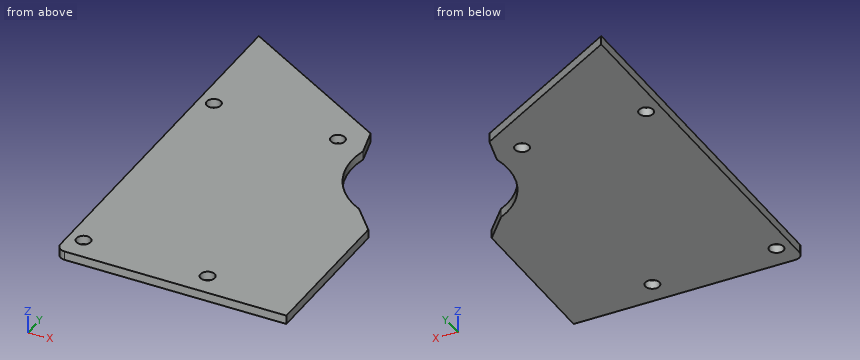
```python
from build123d import *

# Parameters (mm, degrees)
BOSS_EXTRUDE1_DEPTH        = 5
F_16_0_16_DIAMETER_HOLE1_D = 16
FILLET1_R                  = 10


with BuildPart() as part:
    # Sketch1 → Boss-Extrude1 (new, symmetric)
    with BuildSketch(Plane.XY):
        with BuildLine():
            Line((0, 0), (0, 436))
            Line((0, 436), (181, 331.499601277))
            Line((181, 331.499601277), (189.323079198, 299.499601277))
            ThreePointArc((189.323079198, 299.499601277), (195.100872088, 244.235203929), (234.447222331, 205))
            Line((234.447222331, 205), (260, 176))
            Line((260, 176), (260, 0))
            Line((260, 0), (0, 0))
        make_face()
    extrude(amount=BOSS_EXTRUDE1_DEPTH, both=True)

    # Ø16.0 (16) Diameter Hole1 (through all)
    with Locations(Plane.XY.offset(5)):
        with Locations((17, 27), (157, 27), (157, 307), (17, 307)):
            Hole(F_16_0_16_DIAMETER_HOLE1_D / 2)

    # Fillet1
    fillet1_edges = [part.edges().sort_by_distance(p)[0] for p in [
        (0, 0, 0),
    ]]
    fillet(fillet1_edges, radius=FILLET1_R)


solid = part.part
```
Work out the finished part from the listing and answer in its coordinate system (mm). Coordinates: 2 decimals unless noted, no trailing zeros. Write each loop counter-clockwise with the first axis right and the second up, starting at its lowest first coordinate (ties: lowest second). Pieces come first, ordered by that corner, then holes. Notation, with made-up numbers: (-13, -8.5) - (8, -8.5) arc R17 cw to (8, -0.5) - close; hole circle Ø4 at (76.5, -11). An arc over 180 degrees is marked (long way). Answer as a JSON object with one key per item and string values.
Q1. Find section D-D (y = 224). Write down the section's boundary in (x, z), plus the area to 3 significant figures.
Results list:
{"outline": "(0, -5) - (208.74, -5) - (208.74, 5) - (0, 5) - close", "area": "2,090 mm^2"}
Q2. Find section B-B (x = 157). Write down the section's boundary in (y, z), plus the area to 3 significant figures.
Results list:
{"outline": "(0, -5) - (19, -5) - (19, 5) - (0, 5) - close; (35, -5) - (299, -5) - (299, 5) - (35, 5) - close; (315, -5) - (345.36, -5) - (345.36, 5) - (315, 5) - close", "area": "3,130 mm^2"}
Q3. Given pin 1 Ø1.5 at (x, z) = (200, 1) entering from +Y; pin 2 Ø4 at (x, z) = (133, 0.5) entering from +Y, each flat-ended and moving along its own axis, determine where each tip first touches the part or whether it passes through.
Results list:
{"pin 1": "stops at y = 236.6", "pin 2": "stops at y = 360.37"}
Q4. Consider L1, parallel to X at y = 306, z = 4; L2, parallel to Y at x = 156, z = 2.5; L3, parallel to Y at x = 220, z = 2. Determine where each line is inside the solid, lowest interval first. Write a range as from..to.
Results list:
{"L1": "x = 0..9.06, 24.94..149.06, 164.94..187.63", "L2": "y = 0..19.06, 34.94..299.06, 314.94..345.93", "L3": "y = 0..213.75"}
Q5. Find section A-A (y = 27). Write down the section's boundary in (x, z), plus the area to 3 significant figures.
Results list:
{"outline": "(0, -5) - (9, -5) - (9, 5) - (0, 5) - close; (25, -5) - (149, -5) - (149, 5) - (25, 5) - close; (165, -5) - (260, -5) - (260, 5) - (165, 5) - close", "area": "2,280 mm^2"}
Q6. Find section C-C (z = 2). Write down the section's boundary in (x, y).
Results list:
{"outline": "(0, 10) arc R10 ccw to (10, 0) - (260, 0) - (260, 176) - (234.45, 205) arc R83 cw to (189.32, 299.5) - (181, 331.5) - (0, 436) - close; hole circle Ø16 at (17, 27); hole circle Ø16 at (17, 307); hole circle Ø16 at (157, 27); hole circle Ø16 at (157, 307)"}
